Source: CAD feature listing. Evaluate the final solid. Frame: model axes, mm. A direction names the side the tool comes from. Round coordinates to 2 decimals unless told otherwise and drop trailing zeros. Write each loop counter-clockwise with the first axis right and the second up, starting at its lowest first coordinate (ties: lowest second). Pieces come first, ordered by that corner, then holes.
from build123d import *

# Parameters (mm, degrees)
BOSS_EXTRUDE1_DEPTH = 7.9
SHELL1_T            = -3


with BuildPart() as part:
    # Sketch2 → Boss-Extrude1 (new body)
    with BuildSketch(Plane.XY):
        with BuildLine():
            Line((0, 20.9), (-130, 20.9))
            ThreePointArc((-130, 20.9), (-150.9, 0), (-130, -20.9))
            Line((-130, -20.9), (0, -20.9))
            ThreePointArc((0, -20.9), (20.9, 0), (0, 20.9))
        make_face()
    extrude(amount=BOSS_EXTRUDE1_DEPTH)

    # Shell1
    shell1_openings = [part.faces().sort_by_distance(p)[0] for p in [
        (-65, 0, 7.9),
        (-65, 0, 0),
    ]]
    offset(amount=SHELL1_T, openings=shell1_openings, kind=Kind.INTERSECTION)


solid = part.part
1) Section query B-B on z = 6.25. Return the cut outline in (x, y).
Taken from the geometry:
outline: (-130, -20.9) - (0, -20.9) arc R20.9 ccw to (0, 20.9) - (-130, 20.9) arc R20.9 ccw to start; hole (-130, -17.9) - (0, -17.9) arc R17.9 ccw to (0, 17.9) - (-130, 17.9) arc R17.9 ccw to start
2) Pull-direction query (Y, two-part tool) for faces 3 (the face through (17.896, -0.394, 3.895)), 4 (the face through (-64, 17.9, 4)), 5 (the face through (-65.4, -18.5, 0)), 6 (the face through (-66, -20.9, 4)); classes: released by +Y, released by -Y, zero draft, split by the parting line, or undercut.
Taken from the geometry:
face 3: undercut
face 4: undercut
face 5: zero draft
face 6: released by -Y
3) Material intervals for line 1 (Y direction, x = -117, z = 4.75); line 2 (X direction, y = -0.5, z = 2.5); line 3 (X direction, y = -10, z = 5), sorted ascending.
Taken from the geometry:
line 1: y = -20.9 to -17.9, 17.9 to 20.9
line 2: x = -150.89 to -147.89, 17.89 to 20.89
line 3: x = -148.35 to -144.85, 14.85 to 18.35
4) Section query A-A on x = -118. Return the cut outline in (y, z).
Taken from the geometry:
outline: (-20.9, 0) - (-17.9, 0) - (-17.9, 7.9) - (-20.9, 7.9) - close; (17.9, 0) - (20.9, 0) - (20.9, 7.9) - (17.9, 7.9) - close
5) Section query C-C on y = 7. Return the cut outline in (x, z).
Taken from the geometry:
outline: (-149.69, 0) - (-146.47, 0) - (-146.47, 7.9) - (-149.69, 7.9) - close; (16.47, 0) - (19.69, 0) - (19.69, 7.9) - (16.47, 7.9) - close
6) Reachability of faces 1 (the face through (20.895, -0.46, 3.895)), 2 (the face through (-147.896, 0.394, 3.895)) from +Z, -Z, +X, -X, +Y, -Y: full face, straight path, thin tool, end or side. Return the list, or none.
Taken from the geometry:
face 1: +Z, -Z, +X
face 2: +Z, -Z
7) Contact query for flat-ended pins moving along their axis: P1, Ø1, axis at y = -16.5, z = 6.5, coming from the +X side; P2, Ø1, axis at y = -7, z = 2, coming from the -X side. Output: stop coordinate, or through.
Taken from the geometry:
P1: stops at x = 13.45
P2: stops at x = -149.86
